Geometry: final body of the model. Coordinates: model frame, mm. Face numbers are marked on the shaded views. A direction names the side the tool comes from. Give positions to 0.01 mm unless a question says otherwise; leave off trailing zeros. Order: outer loops, then holes, each group sorted by start corner. A loop starts at its lowest first (then second) coordinate and runs counter-clockwise, first axis right, second up. Notation, with made-up numbers: (74.25, 35) -> (130.25, 35) arc R23 ccw to (130.25, 60) -> close; hole circle Ø9 at (-6.5, 32). An arc over 180 degrees is marked (long way). Answer in a Markdown table with one row per item. Add a question column.
Q1. Set-up query: the marked faces 4 and 5. Return all of +Z, -Z, +X, -X, +Y, -Y with unobstructed straight access to the full face (end or side cutting, diameter ignored); none if empty.
Q2. Contact query for a flat-ended pin moving along its axis: P1, Ø5, axis at x = 6.5, z = 100.5, coming from the -Y side. Output: stop coordinate, or through.
Q3. Cut plane A-A on y = -2.5. Return the cut outline in (x, z).
Q4. Cut plane C-C on z = 38.5. Return the cut outline in (x, y), and give its area (3 significant figures).
Q5. Pull-direction query (X, two-part tool) for the marked faces 1, 2 and 3; classes: +X half, -X half, draft (parallel to the pull), parting line (faces both ways), or undercut.
Q6. Line query: line 1 along X through (y, z) = (-21, 86.5); line 2 along Y through (x, z) = (-14, 28.5); line 3 along Y through (x, z) = (-35, 120.5). Output: solid intervals per line, ascending. Write a range as from..to.
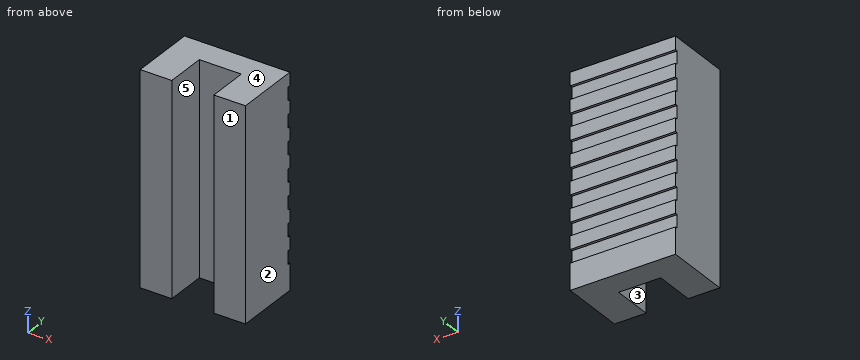
from build123d import *

# Parameters (mm, degrees)
BOSS_EXTRUDE1_DEPTH = 160
SKETCH2_W           = 80
SKETCH2_H           = 10
CUT_EXTRUDE1_DEPTH  = 2
LPATTERN1_COUNT     = 8
LPATTERN1_PITCH     = 20


with BuildPart() as part:
    # Sketch1 → Boss-Extrude1 (new body)
    with BuildSketch(Plane.XY):
        Polygon((0, 6), (0, 25), (-40, 25), (-40, -25), (-16, -25), (-16, 6), align=None)
        Polygon((40, 25), (0, 25), (0, 6), (16, 6), (16, -25), (40, -25), align=None)
    extrude(amount=BOSS_EXTRUDE1_DEPTH)

    # Sketch2 → Cut-Extrude1 (cut)
    with BuildSketch(Plane(origin=(0, 25, 0), x_dir=(1, 0, 0), z_dir=(0, 1, 0))):
        with Locations((0, -25)):
            Rectangle(SKETCH2_W, SKETCH2_H)
    cut_extrude1 = extrude(amount=-CUT_EXTRUDE1_DEPTH, mode=Mode.SUBTRACT)

    # LPattern1: Cut-Extrude1 ×8
    with Locations(*[(0, 0, i * LPATTERN1_PITCH) for i in range(1, LPATTERN1_COUNT)]):
        add(cut_extrude1, mode=Mode.SUBTRACT)


solid = part.part
Completed:
| question | item | result |
|---|---|---|
| 1 | face 4 | +Z, +X, -X, +Y, -Y |
| 1 | face 5 | +Z, -Z, -Y |
| 2 | P1 | stops at y = 6 |
| 3 | outline | (-40, 0) -> (-16, 0) -> (-16, 160) -> (-40, 160) -> close; (16, 0) -> (40, 0) -> (40, 160) -> (16, 160) -> close |
| 4 | outline | (-40, -25) -> (-16, -25) -> (-16, 6) -> (16, 6) -> (16, -25) -> (40, -25) -> (40, 25) -> (-40, 25) -> close |
| 4 | area | 3,010 mm² |
| 5 | face 1 | draft |
| 5 | face 2 | +X half |
| 5 | face 3 | undercut |
| 6 | line 1 | x = -40..-16, 16..40 |
| 6 | line 2 | y = 6..23 |
| 6 | line 3 | y = -25..23 |
